```python
from build123d import *

# Parameters (mm, degrees)
SKETCH2_R           = 14.854735332
SKETCH2_R_2         = 8
BOSS_EXTRUDE1_DEPTH = 28
SKETCH3_R           = 14
CUT_EXTRUDE1_DEPTH  = 16
SKETCH6_W           = 2.60985
SKETCH6_H           = 47.082912009


with BuildPart() as part:
    # Sketch1 → Revolve1 (revolve)
    with BuildSketch(Plane.XY, mode=Mode.PRIVATE) as revolve1_sk:
        Polygon((-43.610341394, 31), (-42.610341394, 31), (-38.591103508, 16), (-33.62957928, 16), (-29.610341394, 31), (-27.610341394, 31), (-27.610341394, 29), (-24.127001892, 16), (-19.021884126, 16), (-16.610341394, 25), (-15.610341394, 25), (-15.610341394, 14), (-43.610341394, 14), align=None)
    revolve(revolve1_sk.sketch.rotate(Axis((-65.147183499, 0, 0), (1, 0, 0)), 90), axis=Axis((-65.147183499, 0, 0), (1, 0, 0)))

    # Sketch2 → Boss-Extrude1 (add, through all)
    with BuildSketch(Plane(origin=(-15.610341394, 0, 0), x_dir=(0, 0, -1), z_dir=(1, 0, 0))):
        Circle(SKETCH2_R)
        Circle(SKETCH2_R_2, mode=Mode.SUBTRACT)
    extrude(amount=-BOSS_EXTRUDE1_DEPTH)

    # Sketch3 → Cut-Extrude1 (cut)
    with BuildSketch(Plane.ZY.offset(43.610341394)):
        Circle(SKETCH3_R)
    extrude(amount=-CUT_EXTRUDE1_DEPTH, mode=Mode.SUBTRACT)

    # Sketch6 → #5 (0.2055) Diameter Hole1 (revolve, cut)
    with BuildSketch(Plane(origin=(-21.548066642, 0.042850676, 15.999942619), x_dir=(0, -0.9999964137036997, 0.0026781672351362563), z_dir=(1, 0, 0))):
        with Locations((1.304925, 23.541456005)):
            Rectangle(SKETCH6_W, SKETCH6_H)
    revolve(axis=Axis((-21.548066642, 0.059857038, 22.349919846), (0, -0.0026781672351362563, -0.9999964137036995)), mode=Mode.SUBTRACT)


solid = part.part
```
The listing builds one solid part. Answer for the finished solid, in the listing's coordinates (mm). A direction names the side the tool comes from. Coordinates: 2 decimals unless noted, no trailing zeros. Write each loop counter-clockwise with the first axis right and the second up, starting at its lowest first coordinate (ties: lowest second). Pieces come first, ordered by that corner, then holes. Notation, with made-up numbers: (11.25, 48) - (42.25, 48) arc R30 ccw to (42.25, 81) - close; hole circle Ø6 at (77.25, -2.75). An arc over 180 degrees is marked (long way). Return JSON: item names as keys, results as strings. Group by question number.
1. A cutting plane is placed at B-B, the plane x = -35.5. Determine the outline of the cut face in (y, z).
2. Given pin 1 (17 mm diameter, centred on y = 0, z = 0, fed in from -X); pin 2 (1.5 mm diameter, centred on x = -18.5, z = -22.5, fed in from -Y) (1 decimal); pin 3 (5 mm diameter, centred on x = -18.5, z = 4, fed in from -Y); pin 4 (1 mm diameter, centred on x = -37, y = 7.5, fed in from +Z), each flat-ended and moving along its own axis, determine where each tip first touches the part or whether it passes through.
3. Straight lines are drawn through the part: L1, parallel to Y at x = -22.75, z = 0; L2, parallel to X at y = 11.5, z = -21.5; L3, parallel to X at y = -21, z = 5. For each, find the intervals that lie inside material, in ascending order.
4. Which of the six approach directions +Z, -Z, +X, -X, +Y, -Y give full straight-line access (tool end or side, diameter ignored) to faces 1 (the cylindrical face through (-22, 16, 0)), 2 (the cylindrical face through (-20.55, -2.38, 11.72)), 3 (the flat face through (-27.61, -6, 6)), 4 (the flat face through (-27.61, 21, 21))?
5. Determine the mould class of faces 5 (the flat face through (-15.61, 6, 6)), 6 (the cylindrical face through (-21.53, -3.06, -7.39)), 7 (the cylindrical face through (-22, -16, 0)), 8 (the cylindrical face through (-16.103, -7.509, 23.846)) for opening direction Y: released by +Y, released by -Y, zero draft, split by the parting line, or undercut.
Ans:
{
 "1": {"outline": "circle Ø32 at (0, 0); hole circle Ø28 at (0, 0)"},
 "2": {"pin 1": "x = -27.61", "pin 2": "through", "pin 3": "y = -24.89", "pin 4": "z = 14.39"},
 "3": {"L1": "-16 to -8, 8 to 16", "L2": "-43.61 to -40.84, -31.38 to -26.37, -16.78 to -15.61", "L3": "-43.61 to -40.09, -32.13 to -25.62, -17.52 to -15.61"},
 "4": {"face 1": "+Y", "face 2": "none", "face 3": "-X", "face 4": "+X"},
 "5": {"face 5": "zero draft", "face 6": "undercut", "face 7": "released by -Y", "face 8": "split by the parting line"}
}
